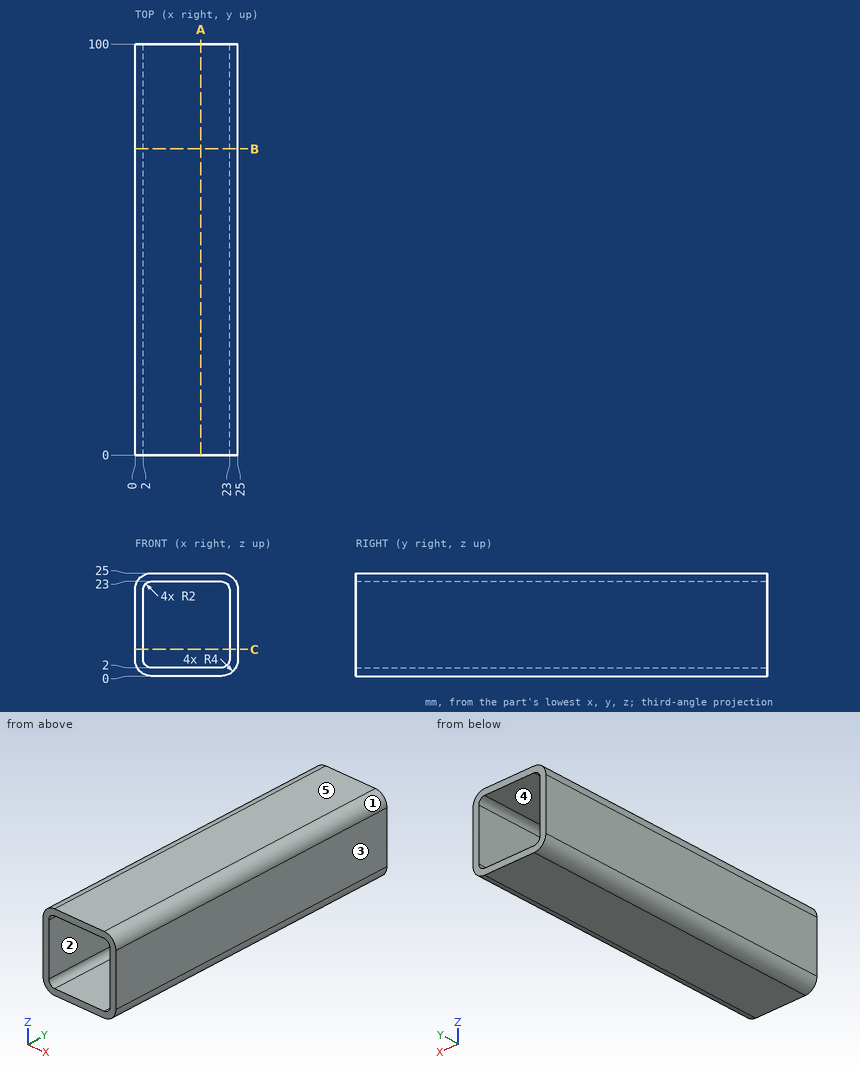
Geometry check sheet. Reference: drawing and pictorial views, mm from the part's lowest x, y, z. A direction names the side the tool comes from. Coordinates: 2 decimals unless noted, no trailing zeros. Order: outer loops, then holes, each group sorted by start corner. A loop starts at its lowest first (then second) coordinate and runs counter-clockwise, first axis right, second up. Notation, with made-up numbers: (-35.5, 66.25) - (-11.5, 66.25) arc R16 cw to (-11.5, 94.25) - close; hole circle Ø4 at (47, 4.25). An arc over 180 degrees is marked (long way). Answer in a Markdown table with one row per item. Add a question column.
1) Set-up check for the marked faces 1 and 2: record each of +Z, -Z, +X, -X, +Y, -Y from which the full face is reachable in a straight line by a thin tool's end or side.
2) Release check for a two-part mould opening along X. For the marked faces 3, 4 and 5 record: +X half, -X half, draft (parallel to the pull), parting line (faces both ways), or undercut.
3) Cross-section at C-C, the plane z = 6.5. Record the cut outline in (x, y), then the cut area to 3 significant figures.
4) Cross-section at B-B, the plane y = 74.5. Record the cut outline in (x, z), then the cut area to 3 significant figures.
5) Cross-section at A-A, the plane x = 16. Record the cut outline in (y, z).
6) Material ranges on line 1 along X through (y, z) = (63.5, 19.5); line 2 along Z through (x, y) = (22.5, 45), recorded low to high. Write a range as [from, to].
Check result:
| question | item | result |
|---|---|---|
| 1 | face 1 | +Z, +X, +Y, -Y |
| 1 | face 2 | +Y, -Y |
| 2 | face 3 | +X half |
| 2 | face 4 | undercut |
| 2 | face 5 | draft |
| 3 | outline | (0, 0) - (2, 0) - (2, 100) - (0, 100) - close; (23, 0) - (25, 0) - (25, 100) - (23, 100) - close |
| 3 | area | 400 mm² |
| 4 | outline | (0, 4) arc R4 ccw to (4, 0) - (21, 0) arc R4 ccw to (25, 4) - (25, 21) arc R4 ccw to (21, 25) - (4, 25) arc R4 ccw to (0, 21) - close; hole (2, 4) arc R2 ccw to (4, 2) - (21, 2) arc R2 ccw to (23, 4) - (23, 21) arc R2 ccw to (21, 23) - (4, 23) arc R2 ccw to (2, 21) - close |
| 4 | area | 174 mm² |
| 5 | outline | (0, 0) - (100, 0) - (100, 2) - (0, 2) - close; (0, 23) - (100, 23) - (100, 25) - (0, 25) - close |
| 6 | line 1 | x = [0, 2], [23, 25] |
| 6 | line 2 | z = [0.29, 2.68], [22.32, 24.71] |
